from build123d import *

# Parameters (mm, degrees)
CHAMFER1_SIZE = 1
CHAMFER2_SIZE = 0.5


with BuildPart() as part:
    # Sketch1 → Revolve1 (revolve)
    with BuildSketch(Plane.XY, mode=Mode.PRIVATE) as revolve1_sk:
        Polygon((486.666563646, -1172.870531067), (486.666563646, -1112.570531067), (481.666563646, -1112.570531067), (481.666563646, -1108.570531067), (471.666563646, -1108.570531067), (471.666563646, -1180.570531067), (475.916563646, -1180.570531067), (475.916563646, -1174.870531067), (477.916563646, -1174.870531067), (477.916563646, -1172.870531067), align=None)
    revolve(revolve1_sk.sketch.rotate(Axis((471.666563646, -1180.570531067, 0), (0, 1, 0)), 90), axis=Axis((471.666563646, -1180.570531067, 0), (0, 1, 0)))

    # Chamfer1
    chamfer1_edges = [part.edges().sort_by_distance(p)[0] for p in [
        (471.666563646, -1112.570531067, 15),
        (471.666563646, -1172.870531067, 15),
        (471.666563646, -1180.570531067, 4.25),
    ]]
    chamfer(chamfer1_edges, length=CHAMFER1_SIZE)

    # Chamfer2
    chamfer2_edges = [part.edges().sort_by_distance(p)[0] for p in [
        (471.666563646, -1108.570531067, 10),
        (471.666563646, -1174.870531067, 6.25),
    ]]
    chamfer(chamfer2_edges, length=CHAMFER2_SIZE)


solid = part.part
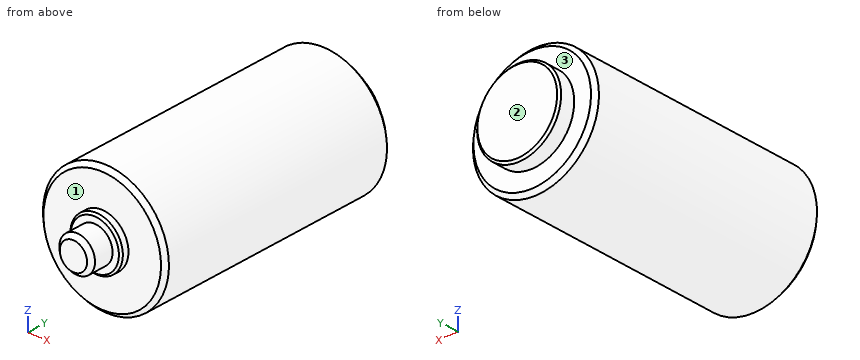
Verification items for the finished model (mm, model axes). Face numbers are marked on the shaded views. A direction names the side the tool comes from. Coordinates: 2 decimals unless noted, no trailing zeros. Order: outer loops, then holes, each group sorted by start corner. A loop starts at its lowest first (then second) coordinate and runs counter-clockwise, first axis right, second up. Notation, with made-up numbers: (54, 33.25) -> (83, 33.25) arc R18 cw to (83, 39.25) -> close; hole circle Ø11 at (30.5, 48). An arc over 180 degrees is marked (long way). Use CSV: the item, a comma, the result in double quotes. Start each with the question number.
Q1. Section check A-A, the plane z = 0. Record the cut outline in (x, y), and give its area (3 significant figures).
Q2. Depth check by flat-ended pin: P1, Ø2, axis at x = 464, y = -1129, coming from the +Z side; P2, Ø4, axis at x = 474, y = -1147, coming from the +Z side; P3, Ø2, axis at x = 479, y = -1118, coming from the +Z side. Enter the tip coordinate at first touch or a pass-through.
Q3. Section check B-B, the plane y = -1169. Record the cut outline in (x, z), and give its area (3 significant figures).
Q4. Thickness scan on line 1 along X through (y, z) = (-1134, 0.5); line 2 along Y through (x, z) = (484.5, -1); line 3 along Y through (x, z) = (479.5, -4.5). Record the ranges inside material, lowest first.
Q5. Tool access check on the marked faces 1, 2 and 3. Record the directions out of +Z, -Z, +X, -X, +Y, -Y that give a thin tool (end or side, any length) a straight path to the whole face; none if there is none.
Returned:
1,outline,"(456.67, -1171.87) -> (457.67, -1172.87) -> (465.42, -1172.87) -> (465.42, -1174.37) -> (465.92, -1174.87) -> (467.42, -1174.87) -> (467.42, -1179.57) -> (468.42, -1180.57) -> (474.92, -1180.57) -> (475.92, -1179.57) -> (475.92, -1174.87) -> (477.42, -1174.87) -> (477.92, -1174.37) -> (477.92, -1172.87) -> (485.67, -1172.87) -> (486.67, -1171.87) -> (486.67, -1113.57) -> (485.67, -1112.57) -> (481.67, -1112.57) -> (481.67, -1109.07) -> (481.17, -1108.57) -> (462.17, -1108.57) -> (461.67, -1109.07) -> (461.67, -1112.57) -> (457.67, -1112.57) -> (456.67, -1113.57) -> close"
1,area,"1,960 mm^2"
2,P1,"stops at z = 13.44"
2,P2,"stops at z = 15"
2,P3,"stops at z = 13.6"
3,outline,"circle Ø30 at (471.67, 0)"
3,area,"707 mm^2"
4,line 1,"x = 456.67 to 486.66"
4,line 2,"y = -1172.87 to -1112.57"
4,line 3,"y = -1172.87 to -1108.57"
5,face 1,"-Y"
5,face 2,"+Z, -Z, +X, -X, +Y"
5,face 3,"+Y"
